Design review of the part built by this model. Coordinates are the model's own, in mm. Round coordinates to 2 decimals unless told otherwise and drop trailing zeros. Order: outer loops, then holes, each group sorted by start corner. A loop starts at its lowest first (then second) coordinate and runs counter-clockwise, first axis right, second up. Notation, with made-up numbers: M 48,54 L 88,54 A24 ccw 88,71 Z; hole C 77.5,55.25 d5. An arc over 180 degrees is marked long. Use a Markdown table: item, result. Add a question column.
(1) Take a section at A-A (y = -12). Write out the cut boundary in (x, z).
(2) Take a section at B-B (z = -2.5). Write out the cut boundary in (x, y), then the cut area to 3 significant figures.
(3) For pin 1 (5 mm diameter, centred on x = 4, z = 31, fed in from -Y); pin 2 (5 mm diameter, centred on x = -0.5, y = -6.5, fed in from +Z); pin 3 (5 mm diameter, centred on x = 5.5, y = -4, fed in from +Z), all flat-tipped, find the tip position at first contact; note any pin that passes through.
(4) To check wall thickness, follow probe 1 along Y at (x, z) = (3.5, 31); probe 2 along Z at (x, y) = (3, -7); probe 3 along Z at (x, y) = (-7, -1.5). State the ranges of each line that lie inside material, in increasing order. Write a range as from..to.
```python
from build123d import *

# Parameters (mm, degrees)
BASE_PROFILE_SKETCH_W          = 50
BASE_PROFILE_SKETCH_H          = 3.464243611
BASE_EXTRUSION_150_DEPTH       = 75
LOUVER_BOSS_DEPTH              = 30
UPPER_CURL_REVOLVE_90DEG_ANGLE = 90
LOWER_CURL_REVOLVE_90DEG_ANGLE = 90
BOTTOM_FILLET_R10_R            = 10
TRIM_CUT_PROFILE_W             = 150
TRIM_CUT_PROFILE_H             = 3.464243611
LOUVER_TRIM_CUT_DEPTH          = 93.33092672


with BuildPart() as part:
    # Base Profile Sketch → Base Extrusion 150 (new, symmetric)
    with BuildSketch(Plane.XY):
        with Locations((0, 1.732121806)):
            Rectangle(BASE_PROFILE_SKETCH_W, BASE_PROFILE_SKETCH_H)
    extrude(amount=BASE_EXTRUSION_150_DEPTH, both=True)

    # Louver Body → Louver Boss (add, symmetric)
    with BuildSketch(Plane.XY):
        with BuildLine():
            Line((-10, 0), (-10, -20))
            ThreePointArc((-10, -20), (4.142135624, -14.142135624), (10, 0))
            Line((10, 0), (-10, 0))
        make_face()
    extrude(amount=LOUVER_BOSS_DEPTH, both=True)

    # Upper Curl Profile → Upper Curl Revolve 90deg (revolve)
    with BuildSketch(Plane.XY.offset(30)):
        with BuildLine():
            Line((10, 0), (-10, 0))
            Line((-10, 0), (-10, -20))
            ThreePointArc((-10, -20), (4.142135624, -14.142135624), (10, 0))
        make_face()
    revolve(axis=Axis((-10, 0, 30), (0, -1, 0)), revolution_arc=UPPER_CURL_REVOLVE_90DEG_ANGLE)

    # Lower Curl Profile → Lower Curl Revolve 90deg (revolve)
    with BuildSketch(Plane(origin=(0, 0, -30), x_dir=(-1, 0, 0), z_dir=(0, 0, -1))):
        with BuildLine():
            Line((10, 0), (-10, 0))
            ThreePointArc((-10, 0), (-4.142135624, -14.142135624), (10, -20))
            Line((10, -20), (10, 0))
        make_face()
    revolve(axis=Axis((-10, -20, -30), (0, 1, 0)), revolution_arc=LOWER_CURL_REVOLVE_90DEG_ANGLE)

    # Bottom Fillet R10
    bottom_fillet_r10_edges = [part.edges().sort_by_distance(p)[0] for p in [
        (10, 0, 0),
        (4.142135624, 0, 44.142135624),
        (4.142135624, 0, -44.142135624),
    ]]
    fillet(bottom_fillet_r10_edges, radius=BOTTOM_FILLET_R10_R)

    # Trim Cut Profile → Louver Trim Cut (cut, through all)
    with BuildSketch(Plane.ZY.offset(25)):
        with Locations((0, 1.732121806)):
            Rectangle(TRIM_CUT_PROFILE_W, TRIM_CUT_PROFILE_H)
    extrude(amount=-LOUVER_TRIM_CUT_DEPTH, mode=Mode.SUBTRACT)


solid = part.part
```
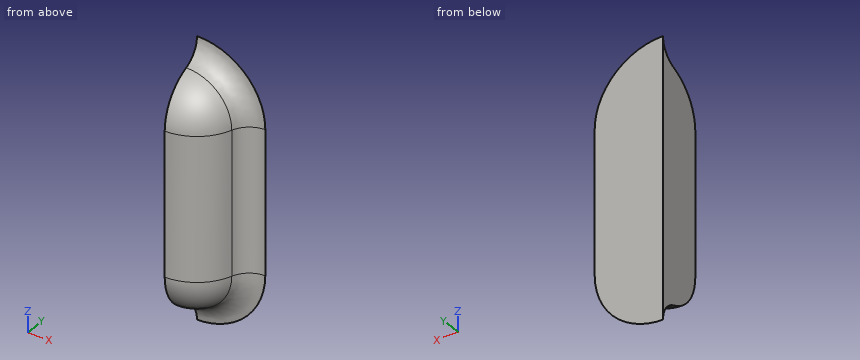
Verdict:
| question | item | result |
|---|---|---|
| 1 | outline | M -10,-46 A16 ccw 6,-30 L 6,30 A16 ccw -10,46 Z |
| 2 | outline | M -10,-20 A20 ccw 8.86,-6.67 A10 cw 18.28,0 L -10,0 Z |
| 2 | area | 326 mm^2 |
| 3 | pin 1 | stops at y = -16.34 |
| 3 | pin 2 | stops at z = 48.27 |
| 3 | pin 3 | stops at z = 47.46 |
| 4 | probe 1 | y = -14.72..0 |
| 4 | probe 2 | z = -43.49..43.49 |
| 4 | probe 3 | z = -52.82..52.82 |
